Can you work these out from the drawing? Everything is in mm from the part's minimum corner. A direction names the side the tool comes from. Coordinates: 2 decimals unless noted, no trailing zeros. Order: outer loops, then holes, each group sorted by start corner. A loop starts at its lowest first (then second) coordinate and runs counter-clockwise, first axis right, second up. Notation, with made-up numbers: (73.5, -14) -> (104.5, -14) arc R18 ccw to (104.5, 10) -> close; hole circle Ø10 at (19.25, 25.5). An arc over 180 degrees is marked (long way). Return JSON: item names as keys, results as strings. Group by question number.
1) Thinking about a two-plate mould opening in Y: for the marked faces 1, 2 and 3, which applies, +Y half, -Y half, draft (parallel to the pull), parting line (faces both ways), or undercut?
2) For pin 1 (8 mm diameter, centred on x = 35.5, z = 15.5, fed in from -Y); pin 2 (4 mm diameter, centred on x = 15.5, z = 5, fed in from -Y); pin 3 (4 mm diameter, centred on x = 17.5, z = 4.5, fed in from -Y), each with a flat end and sliding along its axis, tell me the tip position at first contact or that it passes through.
3) If we section it at A-A, the plane y = 25: Please give me the cut outline in (x, z) (3 decimals), then the cut area to 3 significant figures.
4) If I drill on probe 1 along Y at (x, z) = (25, 10.5) (3 decimals); probe 2 along Y at (x, z) = (25, 7.75) (3 decimals); probe 3 along Z at (x, y) = (10, 38.5), over which ranges is the centre line in solid material (lowest first)? Write a range as from..to.
5) For the marked faces 4 and 5, which set-ups out of +Z, -Z, +X, -X, +Y, -Y let a thin tool reach every point of the face, with its end or its side?
6) If we section it at C-C, the plane z = 1.5: Please give me the cut outline in (x, y) (3 decimals).
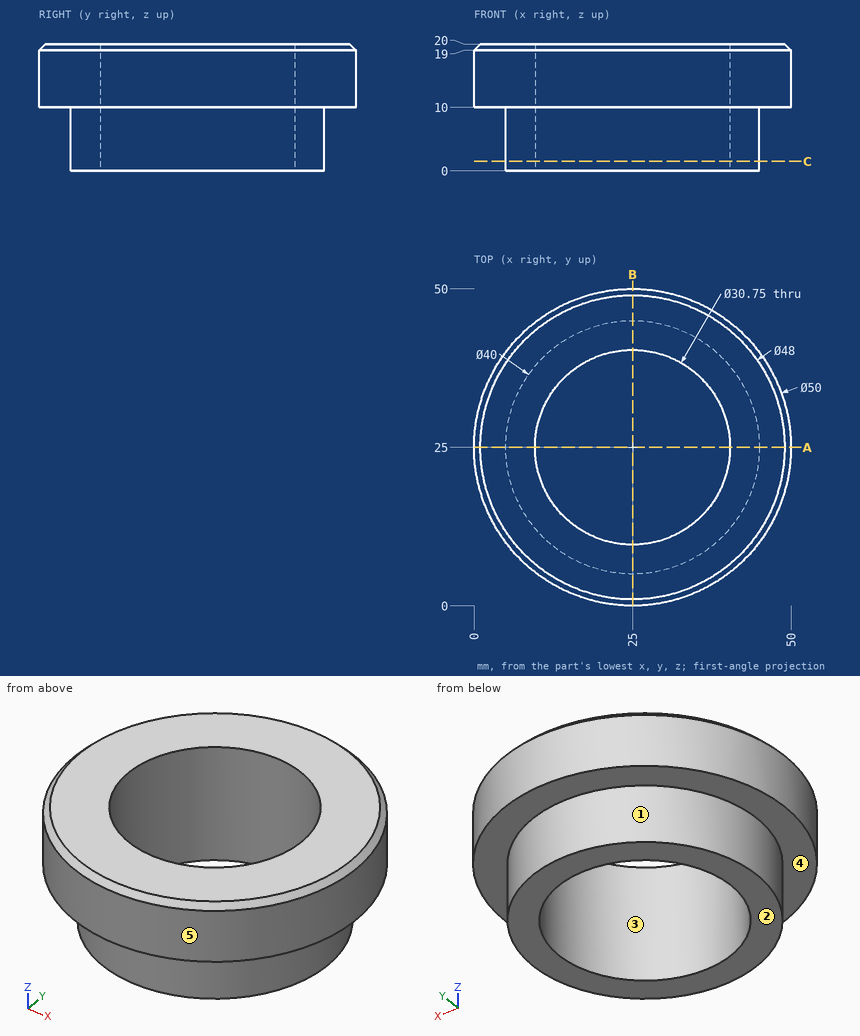
Result sheet:
{
 "1": {"face 1": "parting line", "face 2": "draft", "face 3": "undercut"},
 "2": {"pin 1": "stops at y = 0.86", "pin 2": "stops at y = 6.46", "pin 3": "stops at y = 5.77"},
 "3": {"outline": "(0, 10) -> (5, 10) -> (5, 0) -> (9.625, 0) -> (9.625, 20) -> (1, 20) -> (0, 19) -> close; (40.375, 0) -> (45, 0) -> (45, 10) -> (50, 10) -> (50, 19) -> (49, 20) -> (40.375, 20) -> close", "area": "284 mm2"},
 "4": {"probe 1": "y = 0..9.625, 40.375..50", "probe 2": "y = 5..9.625, 40.375..45", "probe 3": "z = 10..20"},
 "5": {"face 4": "-Z", "face 5": "+Z, -Z"},
 "6": {"outline": "circle Ø40 at (25, 25); hole circle Ø30.75 at (25, 25)"}
}
